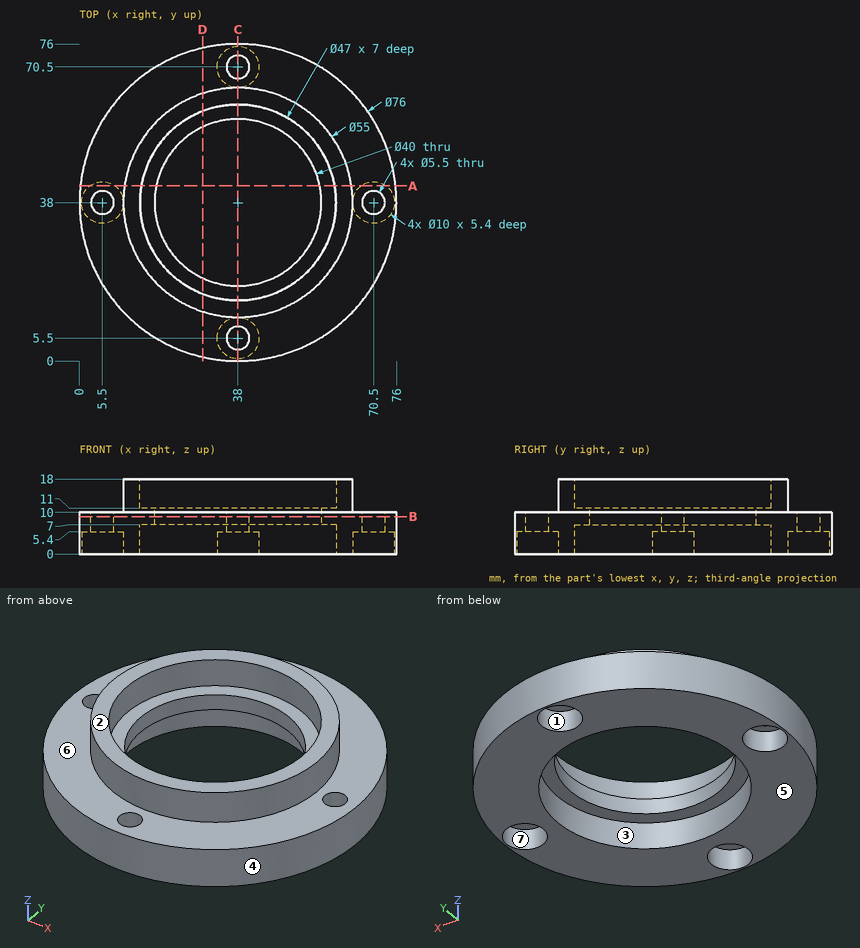
Geometry check sheet. Reference: drawing and pictorial views, mm from the part's lowest x, y, z. A direction names the side the tool comes from. Round coordinates to 2 decimals unless told otherwise and drop trailing zeros. Order: outer loops, then holes, each group sorted by start corner. A loop starts at its lowest first (then second) coordinate and runs counter-clockwise, first axis right, second up.
Q1. Scan lines: L1, parallel to Y at x = 38, z = 3.75; L2, parallel to Y at x = 38, z = 7.1; L3, parallel to Z at x = 38.5, y = 59. Record each from-to range of solid material in increasing order.
Filled sheet:
L1: y = 0 to 0.5, 10.5 to 14.5, 61.5 to 65.5, 75.5 to 76
L2: y = 0 to 2.75, 8.25 to 18, 58 to 67.75, 73.25 to 76
L3: z = 7 to 11
Q2. Cross-section at A-A, the plane y = 42. Enter the section's corners in (x, z), plus the area to 3 significant figures.
Filled sheet:
outline: (0.21, 0) - (2.5, 0) - (2.5, 5.4) - (8.5, 5.4) - (8.5, 0) - (14.84, 0) - (14.84, 7) - (18.4, 7) - (18.4, 11) - (14.84, 11) - (14.84, 18) - (10.79, 18) - (10.79, 10) - (0.21, 10) - close; (57.6, 7) - (61.16, 7) - (61.16, 0) - (67.5, 0) - (67.5, 5.4) - (73.5, 5.4) - (73.5, 0) - (75.79, 0) - (75.79, 10) - (65.21, 10) - (65.21, 18) - (61.16, 18) - (61.16, 11) - (57.6, 11) - close
area: 321 mm2
Q3. Cross-section at D-D, the plane x = 29.5. Enter the section's corners in (y, z).
Filled sheet:
outline: (0.96, 0) - (16.09, 0) - (16.09, 7) - (19.9, 7) - (19.9, 11) - (16.09, 11) - (16.09, 18) - (11.85, 18) - (11.85, 10) - (0.96, 10) - close; (56.1, 7) - (59.91, 7) - (59.91, 0) - (75.04, 0) - (75.04, 10) - (64.15, 10) - (64.15, 18) - (59.91, 18) - (59.91, 11) - (56.1, 11) - close
Q4. Set-up check for the marked faces 5, 6 and 7: record each of +Z, -Z, +X, -X, +Y, -Y from which the full face is reachable in a straight line by a thin tool's end or side.
Filled sheet:
face 5: -Z, +X, -X, +Y, -Y
face 6: +Z
face 7: -Z
Q5. Cross-section at B-B, the plane z = 9. Enter the section's corners in (x, y).
Filled sheet:
outline: circle Ø76 at (38, 38); hole circle Ø5.5 at (5.5, 38); hole circle Ø40 at (38, 38); hole circle Ø5.5 at (38, 5.5); hole circle Ø5.5 at (38, 70.5); hole circle Ø5.5 at (70.5, 38)
Q6. Cross-section at C-C, the plane x = 38. Give the number of separate pieces and of enclosed holes in the cut face, plus the area to 3 significant figures.
Filled sheet:
separate pieces: 4
enclosed holes: 0
area: 223 mm2
Q7. Draft check along Y on the marked faces 1, 2, 3 and 4. Enter one of: pulls with the +Y half, pulls with the -Y half, needs draft (parallel to the pull), parting line crosses it, or undercut.
Filled sheet:
face 1: undercut
face 2: needs draft
face 3: undercut
face 4: parting line crosses it
Q8. Depth check by flat-ended pin: P1, Ø4, axis at y = 20.5, z = 11, coming from the +X side; P2, Ø23.5, axis at x = 40.5, y = 48, coming from the -Z side; P3, Ø7, axis at x = 38, y = 70.5, coming from the +Z side. Enter the tip coordinate at first touch or a pass-through.
Filled sheet:
P1: stops at x = 72.57
P2: stops at z = 7
P3: stops at z = 10
